from build123d import *

# Parameters (mm, degrees)
SKETCH1_R           = 11
BOSS_EXTRUDE1_DEPTH = 15
SKETCH2_R           = 11
SKETCH2_R_2         = 9
CUT_EXTRUDE1_DEPTH  = 5
SKETCH3_R           = 6.5
CUT_EXTRUDE2_DEPTH  = 22.610182785
CHAMFER1_SIZE       = 1


with BuildPart() as part:
    # Sketch1 → Boss-Extrude1 (new body)
    with BuildSketch(Plane.XY):
        Circle(SKETCH1_R)
    extrude(amount=BOSS_EXTRUDE1_DEPTH)

    # Sketch2 → Cut-Extrude1 (cut)
    with BuildSketch(Plane(origin=(0, 0, 0), x_dir=(-1, 0, 0), z_dir=(0, 0, -1))):
        Circle(SKETCH2_R)
        Circle(SKETCH2_R_2, mode=Mode.SUBTRACT)
    extrude(amount=-CUT_EXTRUDE1_DEPTH, mode=Mode.SUBTRACT)

    # Sketch3 → Cut-Extrude2 (cut, through all)
    with BuildSketch(Plane(origin=(0, 0, 0), x_dir=(-1, 0, 0), z_dir=(0, 0, -1))):
        Circle(SKETCH3_R)
    extrude(amount=-CUT_EXTRUDE2_DEPTH, mode=Mode.SUBTRACT)

    # Chamfer1
    chamfer1_edges = [part.edges().sort_by_distance(p)[0] for p in [
        (-11, 0, 15),
        (-11, 0, 5),
        (9, 0, 0),
    ]]
    chamfer(chamfer1_edges, length=CHAMFER1_SIZE)


solid = part.part
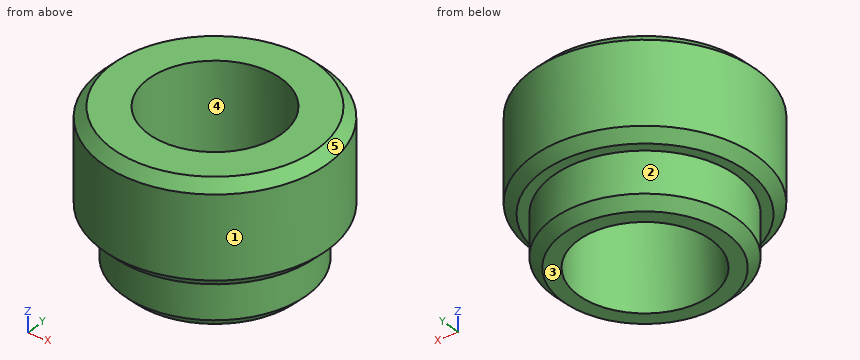
Can you work these out from the model? Positions are in its coordinate system, mm. Face numbers are marked on the shaded views. A direction names the side the tool comes from. Give positions to 0.01 mm unless a question says otherwise; leave off trailing zeros. Loops run counter-clockwise (first coordinate to the right, second up) from the corner with the lowest first, then second, coordinate; pieces in that order, holes last. Notation, with made-up numbers: (44, 40) - (94, 40) arc R18 cw to (94, 75) - close; hole circle Ø7 at (76, -38). An arc over 180 degrees is marked (long way). Return JSON: item names as keys, results as strings.
1. I want a section at D-D on z = 2. Please give me the cut outline in (x, y).
Output values:
{"outline": "circle Ø18 at (0, 0); hole circle Ø13 at (0, 0)"}
2. For the marked faces 1 and 2, which set-ups out of +Z, -Z, +X, -X, +Y, -Y let a thin tool reach every point of the face, with its end or its side?
Output values:
{"face 1": "+Z, -Z", "face 2": "-Z"}
3. I want a section at C-C on z = 11.5. Please give me the cut outline in (x, y).
Output values:
{"outline": "circle Ø22 at (0, 0); hole circle Ø13 at (0, 0)"}
4. I'm going to push flat-ended pins straight in: pin 1 Ø1 at (y, z) = (2, 11) entering from -X; pin 2 Ø4 at (x, z) = (4.5, 11) entering from +Y; pin 3 Ø6 at (x, z) = (-5.5, 8.5) entering from -Y; pin 4 Ø2 at (x, y) = (2, 4.5) entering from +Z. Where does each tip first touch, or does it pass through?
Output values:
{"pin 1": "stops at x = -10.9", "pin 2": "stops at y = 10.71", "pin 3": "stops at y = -10.71", "pin 4": "passes through"}
5. We'd pull the mould along Y, two halves only. Please class the marked faces 3, 4 and 5: +Y half, -Y half, draft (parallel to the pull), parting line (faces both ways), or undercut.
Output values:
{"face 3": "draft", "face 4": "undercut", "face 5": "parting line"}
6. If I drill on line 1 (Y direction, x = 0, z = 7.5); line 2 (X direction, y = -3.75, z = 12); line 3 (X direction, y = -2, z = 3.25), over which ranges is the centre line in solid material (lowest first)?
Output values:
{"line 1": "y = -11 to -6.5, 6.5 to 11", "line 2": "x = -10.34 to -5.31, 5.31 to 10.34", "line 3": "x = -8.77 to -6.18, 6.18 to 8.77"}
7. I want a section at A-A on y = 0. Please give me the cut outline in (x, z), and give its area (3 significant figures).
Output values:
{"outline": "(-11, 6) - (-10, 5) - (-9, 5) - (-9, 1) - (-8, 0) - (-6.5, 0) - (-6.5, 15) - (-10, 15) - (-11, 14) - close; (6.5, 0) - (8, 0) - (9, 1) - (9, 5) - (10, 5) - (11, 6) - (11, 14) - (10, 15) - (6.5, 15) - close", "area": "112 mm²"}
